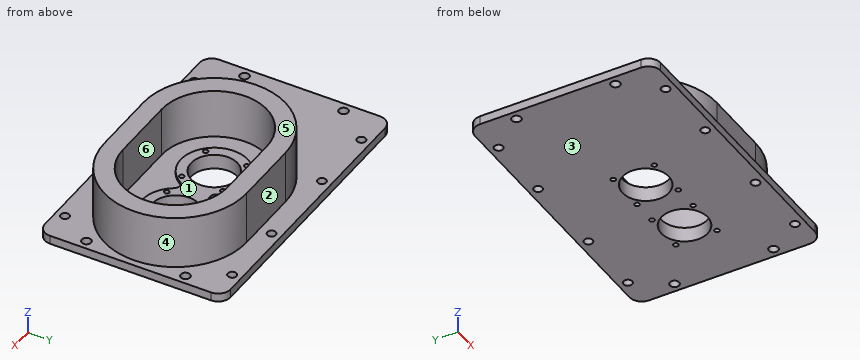
```python
from build123d import *

# Parameters (mm, degrees)
FLANGE_PLATE_SKETCH_W              = 117.5
FLANGE_PLATE_SKETCH_H              = 75
FLANGE_PLATE_DEPTH                 = 3.5
HOUSING_WALL_DEPTH                 = 21.5
HOUSING_CAVITY_DEPTH               = 20
DUAL_BORE_SKETCH_R                 = 9.375
DUAL_BORES_DEPTH                   = 141.823471055
BORE_START                         = 1
BORE_PAD_SKETCH_R                  = 9.375
BORE_PADS_DEPTH                    = 1
BORE_SLOT_SKETCH_R                 = 1
BORE_SLOT_CUT_DEPTH                = 141.684931674
BORE_SLOT_PATTERN_4X_COUNT         = 4
BORE_NOTCH_SKETCH_R                = 1
BORE_NOTCH_CUT_DEPTH               = 141.684931674
BORE_NOTCH_PATTERN_4X_COUNT        = 4
FLANGE_CORNER_FILLETS_R5_R         = 5
FLANGE_EDGE_HOLE_SKETCH_R          = 1.75
FLANGE_EDGE_HOLE_DEPTH             = 142.044319276
FLANGE_EDGE_HOLE_PATTERN_COUNT     = 2
FLANGE_EDGE_HOLE_PATTERN_PITCH     = 27.5
FLANGE_SIDE_HOLE_SKETCH_R          = 1.75
FLANGE_SIDE_HOLES_DEPTH            = 142.044319276
FLANGE_CORNER_HOLE_SKETCH_R        = 1.875
FLANGE_CORNER_HOLES_DEPTH          = 142.044319276
FLANGE_HOLE_MIRROR_COPY_1_SKETCH_R = 1.75
FLANGE_HOLE_MIRROR_COPY_1_DEPTH    = 142.044319276


with BuildPart() as part:
    # Flange Plate Sketch → Flange Plate (new body)
    with BuildSketch(Plane.XY):
        with Locations((58.75, 37.5)):
            Rectangle(FLANGE_PLATE_SKETCH_W, FLANGE_PLATE_SKETCH_H)
    extrude(amount=FLANGE_PLATE_DEPTH)

    # Housing Wall Sketch → Housing Wall (add)
    with BuildSketch(Plane.XY.offset(3.5)):
        with BuildLine():
            Line((59.25, 66.25), (86.25, 66.25))
            ThreePointArc((86.25, 66.25), (115, 37.5), (86.25, 8.75))
            Line((86.25, 8.75), (59.25, 8.75))
            ThreePointArc((59.25, 8.75), (30.5, 37.5), (59.25, 66.25))
        make_face()
    extrude(amount=HOUSING_WALL_DEPTH)

    # Housing Cavity Sketch → Housing Cavity (cut)
    with BuildSketch(Plane.XY.offset(25)):
        with BuildLine():
            Line((86.25, 16.25), (59.25, 16.25))
            ThreePointArc((59.25, 16.25), (38, 37.5), (59.25, 58.75))
            Line((59.25, 58.75), (86.25, 58.75))
            ThreePointArc((86.25, 58.75), (107.5, 37.5), (86.25, 16.25))
        make_face()
    extrude(amount=-HOUSING_CAVITY_DEPTH, mode=Mode.SUBTRACT)

    # Dual Bore Sketch → Dual Bores (cut, through all)
    with BuildSketch(Plane.XY.offset(5)):
        with Locations((59.25, 37.5)):
            Circle(DUAL_BORE_SKETCH_R)
        with Locations((86.25, 37.5)):
            Circle(DUAL_BORE_SKETCH_R)
    extrude(amount=-DUAL_BORES_DEPTH, mode=Mode.SUBTRACT)

    # Bore Pad Sketch → Bore Pads (add)
    with BuildSketch(Plane.XY.offset(5).offset(BORE_START)):
        with BuildLine():
            ThreePointArc((70.640625, 44.745941078), (45.75, 37.5), (70.640625, 30.254058922))
            ThreePointArc((70.640625, 30.254058922), (72.75, 31.412217981), (74.859375, 30.254058922))
            ThreePointArc((74.859375, 30.254058922), (99.75, 37.5), (74.859375, 44.745941078))
            ThreePointArc((74.859375, 44.745941078), (72.75, 43.587782019), (70.640625, 44.745941078))
        make_face()
        with Locations((59.25, 37.5)):
            Circle(BORE_PAD_SKETCH_R, mode=Mode.SUBTRACT)
        with Locations((86.25, 37.5)):
            Circle(BORE_PAD_SKETCH_R, mode=Mode.SUBTRACT)
    extrude(amount=-BORE_PADS_DEPTH)

    # Bore Slot Sketch → Bore Slot Cut (cut, through all)
    with BuildSketch(Plane.XY.offset(6)):
        with Locations((67.558504679, 29.191495321)):
            Circle(BORE_SLOT_SKETCH_R)
    bore_slot_cut = extrude(amount=-BORE_SLOT_CUT_DEPTH, mode=Mode.SUBTRACT)

    # Bore Slot Pattern 4x: Bore Slot Cut ×4 about axis
    bore_slot_pattern_4x_axis = Axis((59.25, 37.5, 0), (0, 0, 1))
    for i in range(1, BORE_SLOT_PATTERN_4X_COUNT):
        add(bore_slot_cut.rotate(bore_slot_pattern_4x_axis, i * 360 / BORE_SLOT_PATTERN_4X_COUNT), mode=Mode.SUBTRACT)

    # Bore Notch Sketch → Bore Notch Cut (cut, through all)
    with BuildSketch(Plane.XY.offset(6)):
        with Locations((94.558504679, 29.191495321)):
            Circle(BORE_NOTCH_SKETCH_R)
    bore_notch_cut = extrude(amount=-BORE_NOTCH_CUT_DEPTH, mode=Mode.SUBTRACT)

    # Bore Notch Pattern 4x: Bore Notch Cut ×4 about axis
    bore_notch_pattern_4x_axis = Axis((86.25, 37.5, 0), (0, 0, 1))
    for i in range(1, BORE_NOTCH_PATTERN_4X_COUNT):
        add(bore_notch_cut.rotate(bore_notch_pattern_4x_axis, i * 360 / BORE_NOTCH_PATTERN_4X_COUNT), mode=Mode.SUBTRACT)

    # Flange Corner Fillets R5
    flange_corner_fillets_r5_edges = [part.edges().sort_by_distance(p)[0] for p in [
        (0, 75, 1.75),
        (117.5, 75, 1.75),
        (117.5, 0, 1.75),
        (0, 0, 1.75),
    ]]
    fillet(flange_corner_fillets_r5_edges, radius=FLANGE_CORNER_FILLETS_R5_R)

    # Flange Edge Hole Sketch → Flange Edge Hole (cut, through all)
    with BuildSketch(Plane.XY.offset(3.5)):
        with Locations((15, 71.25)):
            Circle(FLANGE_EDGE_HOLE_SKETCH_R)
    flange_edge_hole = extrude(amount=-FLANGE_EDGE_HOLE_DEPTH, mode=Mode.SUBTRACT)

    # Flange Edge Hole Pattern: Flange Edge Hole ×2
    with Locations(*[(i * FLANGE_EDGE_HOLE_PATTERN_PITCH, 0, 0) for i in range(1, FLANGE_EDGE_HOLE_PATTERN_COUNT)]):
        add(flange_edge_hole, mode=Mode.SUBTRACT)

    # Flange Side Hole Sketch → Flange Side Holes (cut, through all)
    with BuildSketch(Plane.XY.offset(3.5)):
        with Locations((77.5, 71.25)):
            Circle(FLANGE_SIDE_HOLE_SKETCH_R)
        with Locations((105, 71.25)):
            Circle(FLANGE_SIDE_HOLE_SKETCH_R)
    flange_side_holes = extrude(amount=-FLANGE_SIDE_HOLES_DEPTH, mode=Mode.SUBTRACT)

    # Flange Corner Hole Sketch → Flange Corner Holes (cut, through all)
    with BuildSketch(Plane.XY.offset(3.5)):
        with Locations((113.75, 57.5)):
            Circle(FLANGE_CORNER_HOLE_SKETCH_R)
        with Locations((113.75, 17.5)):
            Circle(FLANGE_CORNER_HOLE_SKETCH_R)
    flange_corner_holes = extrude(amount=-FLANGE_CORNER_HOLES_DEPTH, mode=Mode.SUBTRACT)

    # Flange Hole Mirror: Flange Edge Hole, Flange Side Holes across plane
    add(flange_edge_hole.mirror(Plane.ZX.offset(37.5)), mode=Mode.SUBTRACT)
    add(flange_side_holes.mirror(Plane.ZX.offset(37.5)), mode=Mode.SUBTRACT)

    # Flange Hole Mirror copy 1 sketch → Flange Hole Mirror copy 1 (cut, through all)
    with BuildSketch(Plane(origin=(27.5, 75, 3.5), x_dir=(1, 0, 0), z_dir=(0, 0, 1))):
        with Locations((15, -71.25)):
            Circle(FLANGE_HOLE_MIRROR_COPY_1_SKETCH_R)
    extrude(amount=-FLANGE_HOLE_MIRROR_COPY_1_DEPTH, mode=Mode.SUBTRACT)

    # Corner Hole Mirror: Flange Corner Holes across plane
    add(flange_corner_holes.mirror(Plane(origin=(58.75, 0, 0), x_dir=(0, 0, 1), z_dir=(1, 0, 0))), mode=Mode.SUBTRACT)


solid = part.part
```
Verification items for the finished model (mm, model axes). Face numbers are marked on the shaded views. A direction names the side the tool comes from. Coordinates: 2 decimals unless noted, no trailing zeros. Loops run counter-clockwise (first coordinate to the right, second up) from the corner with the lowest first, then second, coordinate; pieces in that order, holes last. Notation, with made-up numbers: (51.25, 54.25) -> (58.25, 54.25) arc R18 cw to (58.25, 65.25) -> close; hole circle Ø9 at (17.5, 21). An arc over 180 degrees is marked (long way). Put each result on its own line as item: value.
1. Tool access check on the marked faces 1, 2 and 3. Record the directions out of +Z, -Z, +X, -X, +Y, -Y that give a thin tool (end or side, any length) a straight path to the whole face; none if there is none.
Result set:
face 1: +Z
face 2: +Z, +X, -X, +Y
face 3: -Z, +X, -X, +Y, -Y
2. Section check C-C, the plane y = 71.25. Record the boundary of the cut face in (x, z), then the cut area to 3 significant figures.
Result set:
outline: (0.16, 0) -> (13.25, 0) -> (13.25, 3.5) -> (0.16, 3.5) -> close; (16.75, 0) -> (40.75, 0) -> (40.75, 3.5) -> (16.75, 3.5) -> close; (44.25, 0) -> (75.75, 0) -> (75.75, 3.5) -> (44.25, 3.5) -> close; (79.25, 0) -> (103.25, 0) -> (103.25, 3.5) -> (79.25, 3.5) -> close; (106.75, 0) -> (117.34, 0) -> (117.34, 3.5) -> (106.75, 3.5) -> close
area: 361 mm^2
3. Gauge pin test, flat ends, axial feed: P1, Ø4, axis at x = 98.5, z = 13.5, coming from the -Y side; P2, Ø5, axis at y = 10, z = 21.5, coming from the -X side; P3, Ø24.5, axis at x = 59.25, y = 37.5, coming from the +Z side. Record the tip position at first contact, or that the pin passes through.
Result set:
P1: stops at y = 10.64
P2: stops at x = 45.05
P3: stops at z = 6
4. Section check A-A, the plane x = 15. Record the boundary of the cut face in (y, z), then the cut area to 3 significant figures.
Result set:
outline: (0, 0) -> (2, 0) -> (2, 3.5) -> (0, 3.5) -> close; (5.5, 0) -> (69.5, 0) -> (69.5, 3.5) -> (5.5, 3.5) -> close; (73, 0) -> (75, 0) -> (75, 3.5) -> (73, 3.5) -> close
area: 238 mm^2
5. Thickness scan on line 1 (Y direction, x = 87, z = 10.5); line 2 (X direction, y = 71.25, z = 2.3); line 3 (Y direction, x = 94.5, z = 3). Record the ranges inside material, lowest first.
Result set:
line 1: y = 8.76 to 16.26, 58.74 to 66.24
line 2: x = 0.16 to 13.25, 16.75 to 40.75, 44.25 to 75.75, 79.25 to 103.25, 106.75 to 117.34
line 3: y = 0 to 28.19, 30.19 to 33.05, 41.95 to 44.81, 46.81 to 75
6. Mould release check, pull along X, two halves, no side actions. Record for the marked faces 4, 5 and 6: pulls with the +X half, pulls with the -X half, needs draft (parallel to the pull), parting line crosses it, or undercut.
Result set:
face 4: pulls with the +X half
face 5: needs draft
face 6: undercut
7. Section check D-D, the plane y = 17.5. Record the boundary of the cut face in (x, z) (3 decimals).
Result set:
outline: (0, 0) -> (1.875, 0) -> (1.875, 3.5) -> (0, 3.5) -> close; (5.625, 0) -> (111.875, 0) -> (111.875, 3.5) -> (106.903, 3.5) -> (106.903, 25) -> (93.431, 25) -> (93.431, 5) -> (52.069, 5) -> (52.069, 25) -> (38.597, 25) -> (38.597, 3.5) -> (5.625, 3.5) -> close; (115.625, 0) -> (117.5, 0) -> (117.5, 3.5) -> (115.625, 3.5) -> close
8. Section check B-B, the plane z = 19. Record the boundary of the cut face in (x, y), then the cut area to 3 significant figures.
Result set:
outline: (59.25, 8.75) -> (86.25, 8.75) arc R28.75 ccw to (86.25, 66.25) -> (59.25, 66.25) arc R28.75 ccw to start; hole (59.25, 16.25) -> (86.25, 16.25) arc R21.25 ccw to (86.25, 58.75) -> (59.25, 58.75) arc R21.25 ccw to start
area: 1,580 mm^2
